Design review of the part built by this model. Coordinates are the model's own, in mm. A direction names the side the tool comes from. Coordinates: 2 decimals unless noted, no trailing zeros. Loops run counter-clockwise (first coordinate to the right, second up) from the corner with the lowest first, then second, coordinate; pieces in that order, holes last. Notation, with made-up numbers: (69.5, -14) -> (121.5, -14) arc R22 cw to (121.5, 21) -> close; hole circle Ø1 at (70.5, -7.75). An arc over 180 degrees is marked (long way). Answer as a JSON object with one key per item and string values.
```python
from build123d import *

# Parameters (mm, degrees)
SKETCH_2_W          = 2015
SKETCH_2_H          = 235
EXTRUDE_1_DEPTH     = 2
SKETCH_3_W          = 2
SKETCH_3_H          = 235
EXTRUDE_2_DEPTH     = 114
SKETCH_4_W          = 2011
SKETCH_4_H          = 2
EXTRUDE_3_DEPTH     = 40
SKETCH_5_W          = 1150
SKETCH_5_H          = 130
CUT_EXTRUDE_1_DEPTH = 10
SKETCH_6_W          = 2015
SKETCH_6_H          = 42
EXTRUDE_4_DEPTH     = 2
SKETCH_7_W          = 1154
SKETCH_7_H          = 134
SKETCH_7_W_2        = 1150
SKETCH_7_H_2        = 130
EXTRUDE_5_DEPTH     = 15
SKETCH_8_W          = 1154
SKETCH_8_H          = 134
SKETCH_8_W_2        = 1130
SKETCH_8_H_2        = 110
EXTRUDE_6_DEPTH     = 2


with BuildPart() as part:
    # 草图2 → 凸台-拉伸1 (new body)
    with BuildSketch(Plane.XY):
        with Locations((1007.5, 117.5)):
            Rectangle(SKETCH_2_W, SKETCH_2_H)
    extrude(amount=EXTRUDE_1_DEPTH)

    # 草图3 → 凸台-拉伸2 (add)
    with BuildSketch(Plane(origin=(0, 0, 0), x_dir=(-1, 0, 0), z_dir=(0, 0, -1))):
        with Locations((-2014, 117.5)):
            Rectangle(SKETCH_3_W, SKETCH_3_H)
        with Locations((-1, 117.5)):
            Rectangle(SKETCH_3_W, SKETCH_3_H)
    extrude(amount=EXTRUDE_2_DEPTH)

    # 草图4 → 凸台-拉伸3 (add)
    with BuildSketch(Plane(origin=(0, 0, 0), x_dir=(-1, 0, 0), z_dir=(0, 0, -1))):
        with Locations((-1007.5, 234)):
            Rectangle(SKETCH_4_W, SKETCH_4_H)
    extrude(amount=EXTRUDE_3_DEPTH)

    # 草图5 → 切除-拉伸1 (cut)
    with BuildSketch(Plane.XY.offset(2)):
        with Locations((1340, 120)):
            Rectangle(SKETCH_5_W, SKETCH_5_H)
    extrude(amount=-CUT_EXTRUDE_1_DEPTH, mode=Mode.SUBTRACT)

    # 草图6 → 凸台-拉伸4 (add)
    with BuildSketch(Plane.XZ):
        with Locations((1007.5, -19)):
            Rectangle(SKETCH_6_W, SKETCH_6_H)
    extrude(amount=-EXTRUDE_4_DEPTH)

    # 草图7 → 凸台-拉伸5 (add)
    with BuildSketch(Plane(origin=(0, 0, 0), x_dir=(-1, 0, 0), z_dir=(0, 0, -1))):
        with Locations((-1340, 120)):
            Rectangle(SKETCH_7_W, SKETCH_7_H)
        with Locations((-1340, 120)):
            Rectangle(SKETCH_7_W_2, SKETCH_7_H_2, mode=Mode.SUBTRACT)
    extrude(amount=EXTRUDE_5_DEPTH)

    # 草图8 → 凸台-拉伸6 (add)
    with BuildSketch(Plane(origin=(0, 0, -15), x_dir=(-1, 0, 0), z_dir=(0, 0, -1))):
        with Locations((-1340, 120)):
            Rectangle(SKETCH_8_W, SKETCH_8_H)
        with Locations((-1340, 120)):
            Rectangle(SKETCH_8_W_2, SKETCH_8_H_2, mode=Mode.SUBTRACT)
    extrude(amount=-EXTRUDE_6_DEPTH)


solid = part.part
```
1) Clearance check with a flat-ended pin moving along its axis: pin 1 Ø0.6 at (x, y) = (1163, 234) entering from -Z. State where the tip first meets the part, or that it passes through.
Completed:
{"pin 1": "z = -40"}
2) Add section D-D, the plane x = 715.5. Give the boundary of the cut face in (y, z).
Completed:
{"outline": "(0, -40) -> (2, -40) -> (2, 0) -> (233, 0) -> (233, -40) -> (235, -40) -> (235, 2) -> (0, 2) -> close"}
3) Add section C-C, the plane y = 116.5. Give the boundary of the cut face in (x, z).
Completed:
{"outline": "(0, -114) -> (2, -114) -> (2, 0) -> (763, 0) -> (763, -15) -> (775, -15) -> (775, -13) -> (765, -13) -> (765, 2) -> (0, 2) -> close; (1905, -15) -> (1917, -15) -> (1917, 0) -> (2013, 0) -> (2013, -114) -> (2015, -114) -> (2015, 2) -> (1915, 2) -> (1915, -13) -> (1905, -13) -> close"}
4) For faces 1 (the flat face through (1012, 0, -13)), 2 (the flat face through (1343, 178, -13)), 3 (the flat face through (993, 2, -20)), list the 3-axis set-ups (+Z, -Z, +X, -X, +Y, -Y) from which the entire face can be reached by the end or side of a thin tool; tool diameter is ignored.
Completed:
{"face 1": "+Z, -Z, +X, -X, -Y", "face 2": "+Z", "face 3": "-Z"}
5) Wall thickness on probe 1 along X at (y, z) = (131, -6); probe 2 along Y at (x, z) = (1003, -10.5); probe 3 along X at (y, z) = (111, -81.5): over which ranges is each line inside the solid? List them lowest first.
Completed:
{"probe 1": "0 to 2, 763 to 765, 1915 to 1917, 2013 to 2015", "probe 2": "0 to 2, 53 to 55, 185 to 187, 233 to 235", "probe 3": "0 to 2, 2013 to 2015"}
6) Add section B-B, the plane x = 1072.5. Give the boundary of the cut face in (y, z), and give its area (3 significant figures).
Completed:
{"outline": "(0, -40) -> (2, -40) -> (2, 0) -> (53, 0) -> (53, -15) -> (65, -15) -> (65, -13) -> (55, -13) -> (55, 2) -> (0, 2) -> close; (175, -15) -> (187, -15) -> (187, 0) -> (233, 0) -> (233, -40) -> (235, -40) -> (235, 2) -> (185, 2) -> (185, -13) -> (175, -13) -> close", "area": "470 mm²"}
7) Add section A-A, the plane z = -90. Give the boundary of the cut face in (x, y), and give its area (3 significant figures).
Completed:
{"outline": "(0, 0) -> (2, 0) -> (2, 235) -> (0, 235) -> close; (2013, 0) -> (2015, 0) -> (2015, 235) -> (2013, 235) -> close", "area": "940 mm²"}
8) The part is to be moulded in two halves that separate along X. For faces 4 (the flat face through (0, 116, -57)), 5 (the flat face through (2013, 116, -56)), 6 (the flat face through (2015, 116, -55)), say which applies: pulls with the +X half, pulls with the -X half, needs draft (parallel to the pull), parting line crosses it, or undercut.
Completed:
{"face 4": "pulls with the -X half", "face 5": "undercut", "face 6": "pulls with the +X half"}
